Check sheet for the modelled part. Datum: model origin and axes. Units: mm. A direction names the side the tool comes from. Give positions to 0.01 mm unless a question says otherwise; leave off trailing zeros. Write each loop counter-clockwise with the first axis right and the second up, starting at its lowest first coordinate (ties: lowest second). Pieces come first, ordered by that corner, then holes. Notation, with made-up numbers: (44, 54) -> (102, 54) arc R16 ccw to (102, 61) -> close; hole circle Ø9 at (32, 4). An arc over 180 degrees is marked (long way). Use a Markdown table: item, result. Add a question column.
1. Cross-section at B-B (x = -29). Enter the section's corners in (y, z).
2. Set-up check for faces 1 (the flat face through (-27, 0, 14)), 2 (the flat face through (0, 0, 17.5)): record each of +Z, -Z, +X, -X, +Y, -Y from which the full face is reachable in a straight line by a thin tool's end or side.
3. Scan lines: probe 1 along Z at (x, y) = (29, -1.8); probe 2 along X at (y, z) = (-2, 12.5); probe 3 along X at (y, z) = (-1.5, 11). Record each from-to range of solid material in increasing order. Write a range as [from, to].
4. Cross-section at C-C (y = -1). Enter the section's corners in (x, z).
5. Release check for a two-part mould opening along Z. For faces 3 (the flat face through (0, 0, -17.5)), 4 (the flat face through (-27, 0, -11)), 5 (the flat face through (-35, 0, 0)), 6 (the flat face through (31, 0, -11)) record: released by +Z, released by -Z, zero draft, split by the parting line, or undercut.
6. Gauge pin test, flat ends, axial feed: P1, Ø6.5, axis at x = 29, z = -12.5, coming from the +Y side; P2, Ø10.5, axis at x = 29, z = 12.5, coming from the +Y side. Record the tip position at first contact, or that the pin passes through.
7. Cross-section at A-A (z = 12.5). Enter the section's corners in (x, y).
from build123d import *

# Parameters (mm, degrees)
SKETCH_1_W                   = 70
SKETCH_1_H                   = 35
EXTRUDE_1_DEPTH              = 5
CHAMFER_1_SIZE               = 2
HOLE_WIZARD_M4_1_D           = 4.5
HOLE_WIZARD_M4_1_CBORE_D     = 8
HOLE_WIZARD_M4_1_CBORE_DEPTH = 5


with BuildPart() as part:
    # 草图1 → 凸台-拉伸1 (new, symmetric)
    with BuildSketch(Plane(origin=(0, 0, 0), x_dir=(1, 0, 0), z_dir=(0, 1, 0))):
        Rectangle(SKETCH_1_W, SKETCH_1_H)
    extrude(amount=EXTRUDE_1_DEPTH, both=True)

    # 倒角1
    chamfer_1_edges = [part.edges().sort_by_distance(p)[0] for p in [
        (35, 0, 17.5),
        (-35, 0, 17.5),
        (-35, 0, -17.5),
        (35, 0, -17.5),
    ]]
    chamfer(chamfer_1_edges, length=CHAMFER_1_SIZE)

    # M4 六角圆柱头螺钉的柱形沉头孔1 (through all)
    with Locations(Plane(origin=(0, 5, 0), x_dir=(1, 0, 0), z_dir=(0, 1, 0))):
        with Locations((-29, 12.5), (-29, -12.5), (29, 12.5), (29, -12.5)):
            CounterBoreHole(HOLE_WIZARD_M4_1_D / 2, HOLE_WIZARD_M4_1_CBORE_D / 2, HOLE_WIZARD_M4_1_CBORE_DEPTH)


solid = part.part
Worked answers:
| question | item | result |
|---|---|---|
| 1 | outline | (-5, -17.5) -> (5, -17.5) -> (5, -16.5) -> (0, -16.5) -> (0, -14.75) -> (-5, -14.75) -> close; (-5, -10.25) -> (0, -10.25) -> (0, -8.5) -> (5, -8.5) -> (5, 8.5) -> (0, 8.5) -> (0, 10.25) -> (-5, 10.25) -> close; (-5, 14.75) -> (0, 14.75) -> (0, 16.5) -> (5, 16.5) -> (5, 17.5) -> (-5, 17.5) -> close |
| 2 | face 1 | +Y |
| 2 | face 2 | +Z, +X, -X, +Y, -Y |
| 3 | probe 1 | z = [-17.5, -14.75], [-10.25, 10.25], [14.75, 17.5] |
| 3 | probe 2 | x = [-35, -31.25], [-26.75, 26.75], [31.25, 35] |
| 3 | probe 3 | x = [-35, -30.68], [-27.32, 27.32], [30.68, 35] |
| 4 | outline | (-35, -15.5) -> (-33, -17.5) -> (33, -17.5) -> (35, -15.5) -> (35, 15.5) -> (33, 17.5) -> (-33, 17.5) -> (-35, 15.5) -> close; hole circle Ø4.5 at (-29, -12.5); hole circle Ø4.5 at (-29, 12.5); hole circle Ø4.5 at (29, -12.5); hole circle Ø4.5 at (29, 12.5) |
| 5 | face 3 | released by -Z |
| 5 | face 4 | undercut |
| 5 | face 5 | zero draft |
| 5 | face 6 | undercut |
| 6 | P1 | stops at y = 0 |
| 6 | P2 | stops at y = 5 |
| 7 | outline | (-35, -5) -> (-31.25, -5) -> (-31.25, 0) -> (-33, 0) -> (-33, 5) -> (-35, 5) -> close; (-26.75, -5) -> (26.75, -5) -> (26.75, 0) -> (25, 0) -> (25, 5) -> (-25, 5) -> (-25, 0) -> (-26.75, 0) -> close; (31.25, -5) -> (35, -5) -> (35, 5) -> (33, 5) -> (33, 0) -> (31.25, 0) -> close |
